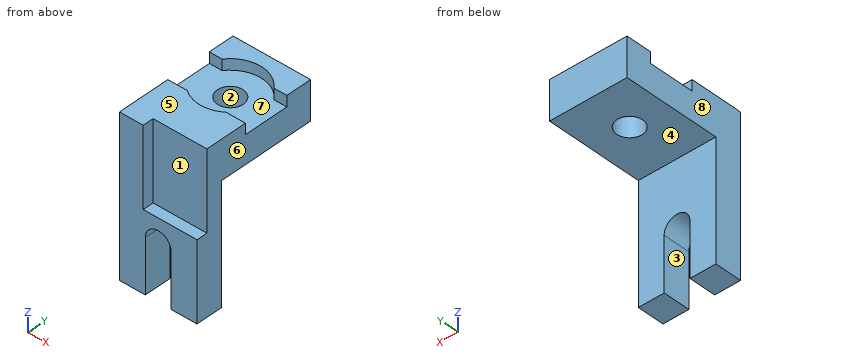
from build123d import *

# Parameters (mm, degrees)
UPRIGHT_BLOCK_PROFILE_W             = 72
UPRIGHT_BLOCK_PROFILE_H             = 90
UPRIGHT_BLOCK_DEPTH                 = 36
SIDE_RECESS_10_DEEP_DEPTH           = 10
BORE_SKETCH_R                       = 12
BORE_24_DEPTH                       = 42
BASE_ARM_SKETCH_W                   = 146
BASE_ARM_SKETCH_H                   = 25
BASE_ARM_146X25_DEPTH               = 72
ARM_SLOT_DEPTH                      = 42
RELIEF_GROOVE_SKETCH_W              = 50
RELIEF_GROOVE_SKETCH_H              = 10
UNDERSIDE_RELIEF_GROOVE_10X50_DEPTH = 73


with BuildPart() as part:
    # Upright Block Profile → Upright Block (new body)
    with BuildSketch(Plane.XY):
        with Locations((36, 45)):
            Rectangle(UPRIGHT_BLOCK_PROFILE_W, UPRIGHT_BLOCK_PROFILE_H)
    extrude(amount=-UPRIGHT_BLOCK_DEPTH)

    # Side Recess Sketch → Side Recess 10 Deep (cut)
    with BuildSketch(Plane.XY):
        with BuildLine():
            Line((0, 66), (12, 66))
            ThreePointArc((12, 66), (36, 78), (60, 66))
            Line((60, 66), (72, 66))
            Line((72, 66), (72, 24))
            Line((72, 24), (54, 24))
            ThreePointArc((54, 24), (36, 18), (18, 24))
            Line((18, 24), (0, 24))
            Line((0, 24), (0, 66))
        make_face()
    extrude(amount=-SIDE_RECESS_10_DEEP_DEPTH, mode=Mode.SUBTRACT)

    # Bore Sketch → Bore Ø24 (cut)
    with BuildSketch(Plane.XY.offset(-10)):
        with Locations((36, 48)):
            Circle(BORE_SKETCH_R)
    extrude(amount=-BORE_24_DEPTH, mode=Mode.SUBTRACT)

    # Base Arm Sketch → Base Arm 146x25 (add)
    with BuildSketch(Plane(origin=(72, 0, 0), x_dir=(0, 0, -1), z_dir=(1, 0, 0))):
        with Locations((73, -12.5)):
            Rectangle(BASE_ARM_SKETCH_W, BASE_ARM_SKETCH_H)
    extrude(amount=-BASE_ARM_146X25_DEPTH)

    # Arm Slot Sketch → Arm Slot (cut)
    with BuildSketch(Plane(origin=(0, 0, 0), x_dir=(1, 0, 0), z_dir=(0, 1, 0))):
        with BuildLine():
            Line((24, 146), (24, 96))
            ThreePointArc((24, 96), (36, 84), (48, 96))
            Line((48, 96), (48, 146))
            Line((48, 146), (24, 146))
        make_face()
    extrude(amount=-ARM_SLOT_DEPTH, mode=Mode.SUBTRACT)

    # Relief Groove Sketch → Underside Relief Groove 10x50 (cut)
    with BuildSketch(Plane.XY):
        with Locations((47, -20)):
            Rectangle(RELIEF_GROOVE_SKETCH_W, RELIEF_GROOVE_SKETCH_H)
    extrude(amount=-UNDERSIDE_RELIEF_GROOVE_10X50_DEPTH, mode=Mode.SUBTRACT)


solid = part.part
Here's how the part is built. I have some questions about the finished solid (model axes, mm). Face numbers are marked on the shaded views. A direction names the side the tool comes from. Round coordinates to 2 decimals unless told otherwise and drop trailing zeros. Write each loop counter-clockwise with the first axis right and the second up, starting at its lowest first coordinate (ties: lowest second). Pieces come first, ordered by that corner, then holes. Notation, with made-up numbers: (34, 87) -> (43, 87) arc R28 ccw to (43, 105) -> close; hole circle Ø2 at (44, 60.5). An arc over 180 degrees is marked (long way). One line per item, written item: value.
1) We'd pull the mould along X, two halves only. Please class the marked faces 5, 6, 7 and 8: released by +X, released by -X, zero draft, split by the parting line, or undercut.
Filled sheet:
face 5: zero draft
face 6: released by +X
face 7: undercut
face 8: released by -X
2) Suppose I cut it at B-B on x = 36. List the corners of the cut face in (y, z) for me, plus the area to 3 significant figures.
Filled sheet:
outline: (-25, -84) -> (0, -84) -> (0, -36) -> (36, -36) -> (36, -10) -> (18, -10) -> (18, 0) -> (-15, 0) -> (-15, -73) -> (-25, -73) -> close; (60, -36) -> (90, -36) -> (90, 0) -> (78, 0) -> (78, -10) -> (60, -10) -> close
area: 3,390 mm2
3) I'm going to push flat-ended pins straight in: pin 1 Ø8 at (y, z) = (-20, -27) entering from +X; pin 2 Ø3 at (x, z) = (17, -121) entering from +Y; pin 3 Ø7.5 at (y, z) = (-18.5, -118) entering from -X; pin 4 Ø15 at (x, z) = (41, -21) entering from -Y. Where does each tip first touch, or does it pass through?
Filled sheet:
pin 1: stops at x = 22
pin 2: stops at y = 0
pin 3: stops at x = 0
pin 4: stops at y = -15
4) If I drill on line 1 (Y direction, x = 36, z = -19); line 2 (Y direction, x = 54, z = -6); line 3 (Z direction, x = 65, y = 19), over which ranges is the centre line in solid material (lowest first)? Write a range as [from, to].
Filled sheet:
line 1: y = [-15, 36], [60, 90]
line 2: y = [-15, 24], [72, 90]
line 3: z = [-36, 0]
5) For the marked faces 1, 2, 3 and 4, which set-ups out of +Z, -Z, +X, -X, +Y, -Y let a thin tool reach every point of the face, with its end or its side?
Filled sheet:
face 1: +Z, +X, -Y
face 2: +Z, -Z
face 3: -Z, +Y, -Y
face 4: -Z, +X, -X, +Y
6) Suppose I cut it at C-C on x = 5. List the corners of the cut face in (y, z) for me, plus the area to 3 significant figures.
Filled sheet:
outline: (-25, -146) -> (0, -146) -> (0, -36) -> (90, -36) -> (90, 0) -> (66, 0) -> (66, -10) -> (24, -10) -> (24, 0) -> (-25, 0) -> close
area: 6,470 mm2
7) Suppose I cut it at A-A on z = -111.5. List the corners of the cut face in (x, y) for me.
Filled sheet:
outline: (0, -25) -> (24, -25) -> (24, 0) -> (0, 0) -> close; (48, -25) -> (72, -25) -> (72, 0) -> (48, 0) -> close
8) Suppose I cut it at D-D on y = 42. List the corners of the cut face in (x, z) for me.
Filled sheet:
outline: (0, -36) -> (25.61, -36) -> (25.61, -10) -> (0, -10) -> close; (46.39, -36) -> (72, -36) -> (72, -10) -> (46.39, -10) -> close
